Print and shaded views of the part. All mm, measured from the part's lowest x, y and z. Round coordinates to 2 decimals unless told otherwise and drop trailing zeros. Write each loop counter-clockwise with the first axis right and the second up, starting at its lowest first coordinate (ties: lowest second). Pieces come first, ordered by that corner, then holes. Notation, with made-up numbers: (-6, 46.5) - (46, 46.5) arc R14 ccw to (46, 70.5) - close; hole circle Ø9 at (23.25, 85.25). An arc over 180 degrees is marked (long way). Put each result on its own line as item: value. Start each with the question number.
Item 1: Cut at B-B (y = 63). Give the cut face in (x, z).
Item 2: Pin check, flat tips, straight feed: pin 1 Ø4 at (x, z) = (20, 11.5) entering from -Y; pin 2 Ø5 at (y, z) = (46.5, 10) entering from +X; pin 3 Ø2 at (x, z) = (59, 19) entering from -Y. Stop position of each tip, or through.
Item 3: Cut at C-C (x = 60). Give the cut face in (y, z), and give its area (3 significant figures).
Item 4: Drill centre lines: line 1 (X direction, y = 36.5, z = 10.5); line 2 (Y direction, x = 45, z = 9.25) (3 decimals); line 3 (X direction, y = 21.5, z = 23.5). Where is each one in solid material? Low to high. Write a range as from..to.
Item 5: Cut at A-A (z = 15.5). Give the cut face in (x, y), and give its area (3 significant figures).
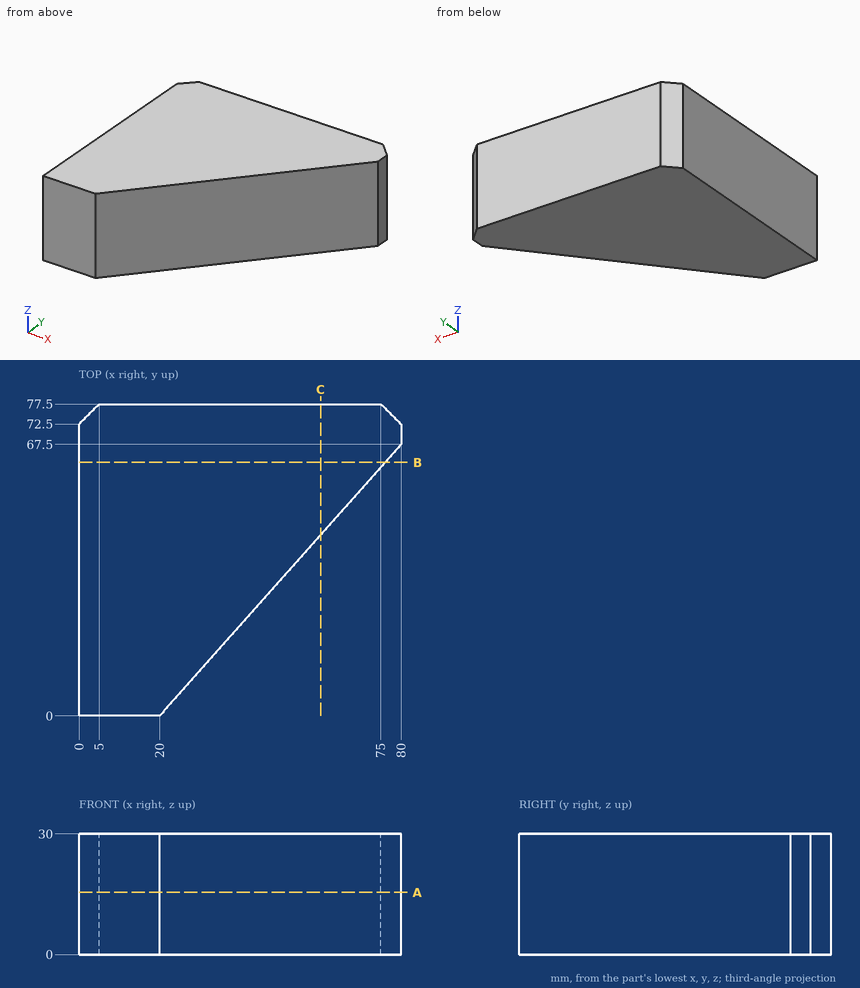
Output values:
1. outline: (0, 0) - (76, 0) - (76, 30) - (0, 30) - close
2. pin 1: y = 0
2. pin 2: x = 63.56
2. pin 3: y = 42.75
3. outline: (45, 0) - (77.5, 0) - (77.5, 30) - (45, 30) - close
3. area: 975 mm2
4. line 1: 0..52.44
4. line 2: 28.125..77.5
4. line 3: 0..39.11
5. outline: (0, 0) - (20, 0) - (80, 67.5) - (80, 72.5) - (75, 77.5) - (5, 77.5) - (0, 72.5) - close
5. area: 4,150 mm2
